```python
from build123d import *

# Parameters (mm, degrees)
GB_T_6728_2002_SQUARE_HOLLOW_SECTION_STE_DEPTH = 100


with BuildPart() as part:
    # Sketch14 → Gb／t 6728—2002 Square hollow section steel 25×2-example.com(1) (new body)
    with BuildSketch(Plane(origin=(0, 0, 0), x_dir=(-1, 0, 0), z_dir=(0, 1, 0))):
        with BuildLine():
            Line((-8.5, -12.5), (8.5, -12.5))
            ThreePointArc((8.5, -12.5), (11.328427125, -11.328427125), (12.5, -8.5))
            Line((12.5, -8.5), (12.5, 8.5))
            ThreePointArc((12.5, 8.5), (11.328427125, 11.328427125), (8.5, 12.5))
            Line((8.5, 12.5), (-8.5, 12.5))
            ThreePointArc((-8.5, 12.5), (-11.328427125, 11.328427125), (-12.5, 8.5))
            Line((-12.5, 8.5), (-12.5, -8.5))
            ThreePointArc((-12.5, -8.5), (-11.328427125, -11.328427125), (-8.5, -12.5))
        make_face()
        with BuildLine():
            Line((-8.5, -10.5), (8.5, -10.5))
            ThreePointArc((8.5, -10.5), (9.914213562, -9.914213562), (10.5, -8.5))
            Line((10.5, -8.5), (10.5, 8.5))
            ThreePointArc((10.5, 8.5), (9.914213562, 9.914213562), (8.5, 10.5))
            Line((8.5, 10.5), (-8.5, 10.5))
            ThreePointArc((-8.5, 10.5), (-9.914213562, 9.914213562), (-10.5, 8.5))
            Line((-10.5, 8.5), (-10.5, -8.5))
            ThreePointArc((-10.5, -8.5), (-9.914213562, -9.914213562), (-8.5, -10.5))
        make_face(mode=Mode.SUBTRACT)
    extrude(amount=GB_T_6728_2002_SQUARE_HOLLOW_SECTION_STE_DEPTH)


solid = part.part
```
Geometry: final body of the model. Coordinates: model frame, mm. A direction names the side the tool comes from. Round coordinates to 2 decimals unless told otherwise and drop trailing zeros. Order: outer loops, then holes, each group sorted by start corner. A loop starts at its lowest first (then second) coordinate and runs counter-clockwise, first axis right, second up. Notation, with made-up numbers: (86, 18.25) - (130, 18.25) arc R22 cw to (130, 35.25) - close; hole circle Ø3 at (-3, 34). An arc over 180 degrees is marked (long way). Use CSV: the item, a comma, the result in double quotes. Start each with the question number.
Q1. Material intervals for line 1 along Z through (x, y) = (3.5, 68.5); line 2 along X through (y, z) = (30, -11), sorted ascending. Write a range as from..to.
Q2. Mould query, pull axis X, two halves, no side actions, for faces 3 (the face through (-10.5, 49, 0)), 4 (the face through (-9.9, 49.3, -9.93)), 5 (the face through (12.5, 49, 0)), 6 (the face through (0, 49, 12.5)). Classes: +X half, -X half, draft (parallel to the pull), parting line (faces both ways), or undercut.
Q3. Section query A-A (y = 31). Return loops of the section in (x, z), and give its area (3 significant figures).
Q4. Section query B-B (x = 2.75). Return loops of the section in (y, z).
Q5. Section query C-C (z = -4.5). Return loops of the section in (x, y).
Q6. First-contact query: pin 1 (2 mm diameter, centred on x = -9, z = -6.5, fed in from -Y); pin 2 (5 mm diameter, centred on y = 50, z = 9.5, fed in from +X). Flat tips, straight axial feed; report the tip coordinate or a pass-through.
Q7. Access query for faces 1 (the face through (0, 49, -10.5)), 2 (the face through (-12.5, 49, 0)). Directions: +Z, -Z, +X, -X, +Y, -Y. A direction counts if a zero-diameter tool reaches every point of the face in a straight line with its end or side. Return the directions, or none.
Result set:
1,line 1,"z = -12.5..-10.5, 10.5..12.5"
1,line 2,"x = -11.62..11.62"
2,face 3,"undercut"
2,face 4,"undercut"
2,face 5,"+X half"
2,face 6,"draft"
3,outline,"(-12.5, -8.5) arc R4 ccw to (-8.5, -12.5) - (8.5, -12.5) arc R4 ccw to (12.5, -8.5) - (12.5, 8.5) arc R4 ccw to (8.5, 12.5) - (-8.5, 12.5) arc R4 ccw to (-12.5, 8.5) - close; hole (-10.5, -8.5) arc R2 ccw to (-8.5, -10.5) - (8.5, -10.5) arc R2 ccw to (10.5, -8.5) - (10.5, 8.5) arc R2 ccw to (8.5, 10.5) - (-8.5, 10.5) arc R2 ccw to (-10.5, 8.5) - close"
3,area,"174 mm2"
4,outline,"(0, -12.5) - (100, -12.5) - (100, -10.5) - (0, -10.5) - close; (0, 10.5) - (100, 10.5) - (100, 12.5) - (0, 12.5) - close"
5,outline,"(-12.5, 0) - (-10.5, 0) - (-10.5, 100) - (-12.5, 100) - close; (10.5, 0) - (12.5, 0) - (12.5, 100) - (10.5, 100) - close"
6,pin 1,"passes through"
6,pin 2,"stops at x = 12.5"
7,face 1,"+Y, -Y"
7,face 2,"+Z, -Z, -X, +Y, -Y"
